CAD build for the part. Positions are in the model's coordinates, mm. Face numbers are marked on the shaded views. A direction names the side the tool comes from. Round coordinates to 2 decimals unless told otherwise and drop trailing zeros. Order: outer loops, then holes, each group sorted by start corner. A loop starts at its lowest first (then second) coordinate and runs counter-clockwise, first axis right, second up. Notation, with made-up numbers: (65.5, 46.25) -> (108.5, 46.25) arc R21 cw to (108.5, 66.25) -> close; hole circle Ø4 at (-31.75, 47). An arc over 180 degrees is marked (long way). Answer as CSV lines item,"result". Start each with the question number.
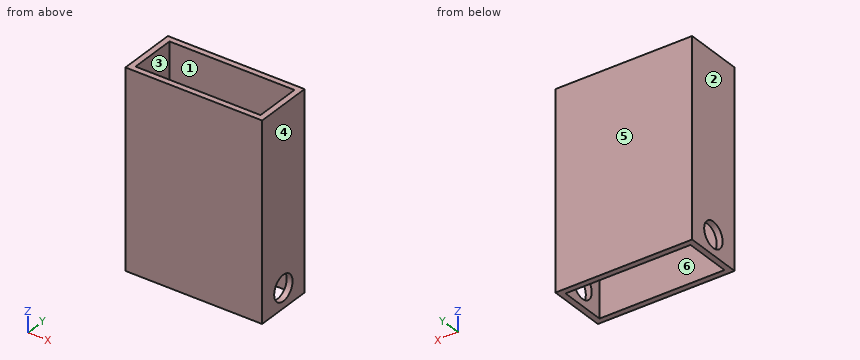
from build123d import *

# Parameters (mm, degrees)
SKETCH_1_W          = 70
SKETCH_1_H          = 30
EXTRUDE_1_DEPTH     = 100
SHELL_1_T           = -3
SKETCH_2_R          = 6.5
CUT_EXTRUDE_2_DEPTH = 100


with BuildPart() as part:
    # 草图1 → 凸台-拉伸1 (new body)
    with BuildSketch(Plane.XY):
        with Locations((35, 15)):
            Rectangle(SKETCH_1_W, SKETCH_1_H)
    extrude(amount=EXTRUDE_1_DEPTH)

    # 抽壳1
    shell_1_openings = [part.faces().sort_by_distance(p)[0] for p in [
        (35, 15, 100),
        (35, 15, 0),
    ]]
    offset(amount=SHELL_1_T, openings=shell_1_openings, kind=Kind.INTERSECTION)

    # 草图2 → 切除-拉伸2 (cut)
    with BuildSketch(Plane.ZY):
        with Locations((10, 15)):
            Circle(SKETCH_2_R)
    extrude(amount=-CUT_EXTRUDE_2_DEPTH, mode=Mode.SUBTRACT)


solid = part.part
Item 1: Band-saw the part on B-B, the plane x = 59. Give the cut face in (y, z), and give its area (3 significant figures).
Item 2: Tool access for the marked faces 5 and 6: list every direction of +Z, -Z, +X, -X, +Y, -Y with a clear straight run to the whole face (end or side of a thin tool).
Item 3: Band-saw the part on A-A, the plane y = 12.5. Give the cut face in (x, z).
Item 4: Probe line 1 (Y direction, x = 52, z = 87.5); line 2 (X direction, y = 8.25, z = 55.5); line 3 (Y direction, x = 1.05, z = 10). List the from-to ranges inside material, lowest first.
Item 5: Pin check, flat tips, straight feed: pin 1 (4 mm diameter, centred on y = 26.5, z = 68, fed in from -X); pin 2 (8 mm diameter, centred on y = 15, z = 10, fed in from +X). Stop position of each tip, or through.
Item 6: Band-saw the part on C-C, the plane z = 72. Give the cut face in (x, y), and give its area (3 significant figures).
Item 7: Mould opens along X. For the marked faces 1, 2, 3 and 4 say: released by +X, released by -X, zero draft, split by the parting line, or undercut.
Item 8: Band-saw the part on D-D, the plane z = 10. Give the cut face in (x, y).
Values:
1,outline,"(0, 0) -> (3, 0) -> (3, 100) -> (0, 100) -> close; (27, 0) -> (30, 0) -> (30, 100) -> (27, 100) -> close"
1,area,"600 mm²"
2,face 5,"+Z, -Z, +X, -X, +Y"
2,face 6,"+Z, -Z"
3,outline,"(0, 0) -> (3, 0) -> (3, 4) -> (0, 4) -> close; (0, 16) -> (3, 16) -> (3, 100) -> (0, 100) -> close; (67, 0) -> (70, 0) -> (70, 4) -> (67, 4) -> close; (67, 16) -> (70, 16) -> (70, 100) -> (67, 100) -> close"
4,line 1,"0 to 3, 27 to 30"
4,line 2,"0 to 3, 67 to 70"
4,line 3,"0 to 8.5, 21.5 to 30"
5,pin 1,"x = 0"
5,pin 2,"through"
6,outline,"(0, 0) -> (70, 0) -> (70, 30) -> (0, 30) -> close; hole (3, 3) -> (67, 3) -> (67, 27) -> (3, 27) -> close"
6,area,"564 mm²"
7,face 1,"undercut"
7,face 2,"released by -X"
7,face 3,"undercut"
7,face 4,"released by +X"
8,outline,"(0, 0) -> (70, 0) -> (70, 8.5) -> (67, 8.5) -> (67, 3) -> (3, 3) -> (3, 8.5) -> (0, 8.5) -> close; (0, 21.5) -> (3, 21.5) -> (3, 27) -> (67, 27) -> (67, 21.5) -> (70, 21.5) -> (70, 30) -> (0, 30) -> close"
